Check sheet for the modelled part. Datum: model origin and axes. Units: mm. A direction names the side the tool comes from. Coordinates: 2 decimals unless noted, no trailing zeros. Loops run counter-clockwise (first coordinate to the right, second up) from the corner with the lowest first, then second, coordinate; pieces in that order, holes last. Notation, with made-up numbers: (11, 73) - (22, 73) arc R15 ccw to (22, 91) - close; hole circle Ø2 at (-17, 70.25). An arc over 180 degrees is marked (long way). Use a Markdown table: item, result. Add a question column.
1) Tool access check on faces 1 (the flat face through (38, 12, 0)), 2 (the flat face through (52, 7.5, 0)), 3 (the flat face through (-2, 2.5, 0)), 4 (the flat face through (3, 10, 0)). Record the directions out of +Z, -Z, +X, -X, +Y, -Y that give a thin tool (end or side, any length) a straight path to the whole face; none if there is none.
2) Sectioned sample at A-A, the plane z = 0. State how many separate pieces and enclosed holes the cut face has, then the cut area to 3 significant figures.
3) Draft check along X on faces 5 (the cylindrical face through (51.464, 1.232, -0.325)), 6 (the cylindrical face through (0.45, 8.73, 1.43)), 7 (the flat face through (47, 5, 0)), 8 (the flat face through (52, 2.5, 0)). Enter one of: pulls with the +X half, pulls with the -X half, needs draft (parallel to the pull), parting line crosses it, or undercut.
4) Thickness scan on line 1 (X direction, y = 1.05, z = 0); line 2 (Z direction, x = 50, y = 1); line 3 (Y direction, x = -1.5, z = 5.75). Record the ranges inside material, lowest first.
5) Sectioned sample at B-B, the plane y = 8.75. Enter the section's corners in (x, z).
6) Go/stop test with flat-tipped pins: P1, Ø6, axis at x = 1.5, z = 0.5, coming from the +Y side; P2, Ø2, axis at y = 7, z = 1, coming from the -X side; P3, Ø2.5, axis at y = 4, z = 2, coming from the +X side. Record where each tip stops, or that it passes through.
7) Sectioned sample at D-D, the plane y = 1. Enter the section's corners in (x, z), then the cut area to 3 significant figures.
8) Sectioned sample at C-C, the plane x = 25. Enter the section's corners in (y, z), then the cut area to 3 significant figures.
from build123d import *

# Parameters (mm, degrees)
SKETCH1_R           = 1.5
BOSS_EXTRUDE1_DEPTH = 10
SKETCH2_W           = 9
SKETCH2_H           = 5
CUT_EXTRUDE1_DEPTH  = 24.832750576
SKETCH3_W           = 12
SKETCH3_H           = 5
BOSS_EXTRUDE2_DEPTH = 32
SKETCH5_W           = 26
SKETCH5_H           = 6
SKETCH5_H_2         = 2.5
BOSS_EXTRUDE6_DEPTH = 12
SKETCH6_R           = 3
CUT_EXTRUDE2_DEPTH  = 59.840887145


with BuildPart() as part:
    # Sketch1 → Boss-Extrude1 (new body)
    with BuildSketch(Plane(origin=(0, 0, 0), x_dir=(1, 0, 0), z_dir=(0, 1, 0))):
        with BuildLine():
            Line((0, 6), (12, 6))
            ThreePointArc((12, 6), (18, 0), (12, -6))
            Line((12, -6), (0, -6))
            ThreePointArc((0, -6), (-6, 0), (0, 6))
        make_face()
        with Locations(Location((0, 0, 0), (0, 0, 270))):
            Circle(SKETCH1_R, mode=Mode.SUBTRACT)
    extrude(amount=BOSS_EXTRUDE1_DEPTH)

    # Sketch2 → Cut-Extrude1 (cut, through all)
    with BuildSketch(Plane.XY.offset(6)):
        with Locations((-1.5, 5)):
            Rectangle(SKETCH2_W, SKETCH2_H)
        with Locations((13.5, 5)):
            Rectangle(SKETCH2_W, SKETCH2_H)
    extrude(amount=-CUT_EXTRUDE1_DEPTH, mode=Mode.SUBTRACT)

    # Sketch3 → Boss-Extrude2 (add)
    with BuildSketch(Plane(origin=(9, 0, 0), x_dir=(0, 0, -1), z_dir=(1, 0, 0))):
        with Locations((0, 5)):
            Rectangle(SKETCH3_W, SKETCH3_H)
    extrude(amount=BOSS_EXTRUDE2_DEPTH)

    # Mirror1: part across plane


with BuildPart() as part_1:
    add(part.part)
    add(part.part.mirror(Plane(origin=(25, 0, 0), x_dir=(0, 0, 1), z_dir=(1, 0, 0))))

    # Sketch5 → Boss-Extrude6 (add)
    with BuildSketch(Plane.XY.offset(6)):
        with Locations((25, 10.5)):
            Rectangle(SKETCH5_W, SKETCH5_H)
        with Locations((25, 1.25)):
            Rectangle(SKETCH5_W, SKETCH5_H_2)
    extrude(amount=-BOSS_EXTRUDE6_DEPTH)

    # Sketch6 → Cut-Extrude2 (cut, through all)
    with BuildSketch(Plane.XY.offset(6)):
        with Locations((25, 9.5)):
            Circle(SKETCH6_R)
    extrude(amount=-CUT_EXTRUDE2_DEPTH, mode=Mode.SUBTRACT)


solid = part_1.part
Solved:
| question | item | result |
|---|---|---|
| 1 | face 1 | +Z, -Z, +X, +Y |
| 1 | face 2 | +Z, -Z, +X |
| 1 | face 3 | +Z, -Z, -X |
| 1 | face 4 | +Z, -Z, -X, +Y |
| 2 | separate pieces | 5 |
| 2 | enclosed holes | 1 |
| 2 | area | 563 mm2 |
| 3 | face 5 | undercut |
| 3 | face 6 | undercut |
| 3 | face 7 | pulls with the +X half |
| 3 | face 8 | needs draft |
| 4 | line 1 | x = -6 to -1.5, 1.5 to 48.5, 51.5 to 56 |
| 4 | line 2 | z = -6 to -1.5, 1.5 to 6 |
| 4 | line 3 | y = 0 to 2.5, 7.5 to 10 |
| 5 | outline | (0, -6) - (22.1, -6) - (22.1, 6) - (0, 6) arc R6 ccw to start; (27.9, -6) - (50, -6) arc R6 ccw to (50, 6) - (27.9, 6) - close; hole circle Ø3 at (0, 0); hole circle Ø3 at (50, 0) |
| 6 | P1 | stops at y = 10 |
| 6 | P2 | stops at x = -6 |
| 6 | P3 | stops at x = 47 |
| 7 | outline | (0, -6) - (50, -6) arc R6 ccw to (50, 6) - (0, 6) arc R6 ccw to start; hole circle Ø3 at (0, 0); hole circle Ø3 at (50, 0) |
| 7 | area | 699 mm2 |
| 8 | outline | (0, -6) - (6.5, -6) - (6.5, 6) - (0, 6) - close; (12.5, -6) - (13.5, -6) - (13.5, 6) - (12.5, 6) - close |
| 8 | area | 90.0 mm2 |
